Read the model definition and answer for the solid it produces. Units are mm, in the model's axes. Face numbers are marked on the shaded views. A direction names the side the tool comes from. Coordinates: 2 decimals unless noted, no trailing zeros. Loops run counter-clockwise (first coordinate to the right, second up) from the corner with the lowest first, then second, coordinate; pieces in that order, holes last.
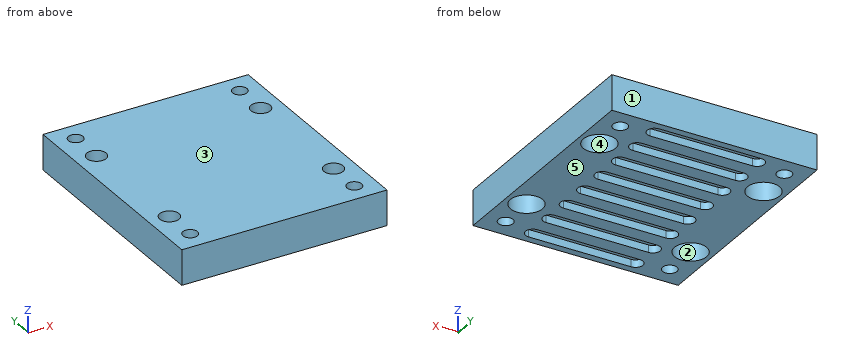
from build123d import *

# Parameters (mm, degrees)
SKETCH_1_W                     = 70
SKETCH_1_H                     = 80
EXTRUDE_1_DEPTH                = 12
HOLE_WIZARD_M6_1_D             = 5
HOLE_WIZARD_M6_1_2_D           = 6.6
HOLE_WIZARD_M6_1_2_CBORE_D     = 11
HOLE_WIZARD_M6_1_2_CBORE_DEPTH = 6.4
CUT_EXTRUDE_1_DEPTH            = 2.5
PATTERN_LINEAR_1_COUNT         = 8
PATTERN_LINEAR_1_PITCH         = 10


with BuildPart() as part:
    # 草图1 → 凸台-拉伸1 (new body)
    with BuildSketch(Plane.XY):
        Rectangle(SKETCH_1_W, SKETCH_1_H)
    extrude(amount=EXTRUDE_1_DEPTH)

    # Hole Wizard M6 _1 (through all)
    with Locations(Plane(origin=(0, 0, 0), x_dir=(-1, 0, 0), z_dir=(0, 0, -1))):
        with Locations((-28, -33), (-28, 33), (28, 33), (28, -33)):
            Hole(HOLE_WIZARD_M6_1_D / 2)

    # Hole Wizard M6 _1 2 (through all)
    with Locations(Plane(origin=(0, 0, 0), x_dir=(-1, 0, 0), z_dir=(0, 0, -1))):
        with Locations((-28, -21), (-28, 21), (28, -21), (28, 21)):
            CounterBoreHole(HOLE_WIZARD_M6_1_2_D / 2, HOLE_WIZARD_M6_1_2_CBORE_D / 2, HOLE_WIZARD_M6_1_2_CBORE_DEPTH)

    # 草图6 → 切除-拉伸1 (cut)
    with BuildSketch(Plane(origin=(0, 0, 0), x_dir=(-1, 0, 0), z_dir=(0, 0, -1))):
        with BuildLine():
            Line((17.5, 32.5), (-17.5, 32.5))
            ThreePointArc((-17.5, 32.5), (-20, 35), (-17.5, 37.5))
            Line((-17.5, 37.5), (17.5, 37.5))
            ThreePointArc((17.5, 37.5), (20, 35), (17.5, 32.5))
        make_face()
    cut_extrude_1 = extrude(amount=-CUT_EXTRUDE_1_DEPTH, mode=Mode.SUBTRACT)

    # 阵列(线性)1: 切除-拉伸1 ×8
    with Locations(*[(0, -i * PATTERN_LINEAR_1_PITCH, 0) for i in range(1, PATTERN_LINEAR_1_COUNT)]):
        add(cut_extrude_1, mode=Mode.SUBTRACT)


solid = part.part
Q1. Flat-ended cylindrical pins translate along their axes: pin 1 Ø2.5 at (x, y) = (7, 24) entering from -Z; pin 2 Ø3 at (x, y) = (28, 33) entering from -Z. Find the tip coordinate at first contact, or state that the pin passes through.
Findings below:
pin 1: stops at z = 2.5
pin 2: passes through
Q2. Which of the six approach directions +Z, -Z, +X, -X, +Y, -Y give full straight-line access (tool end or side, diameter ignored) to the marked faces 4 and 5?
Findings below:
face 4: -Z
face 5: -Z, +X, -X, +Y, -Y
Q3. A cutting plane is placed at B-B (x = 28). Give the vertices of the cut face in (y, z).
Findings below:
outline: (-40, 0) - (-35.5, 0) - (-35.5, 12) - (-40, 12) - close; (-30.5, 0) - (-26.5, 0) - (-26.5, 6.4) - (-24.3, 6.4) - (-24.3, 12) - (-30.5, 12) - close; (-17.7, 6.4) - (-15.5, 6.4) - (-15.5, 0) - (15.5, 0) - (15.5, 6.4) - (17.7, 6.4) - (17.7, 12) - (-17.7, 12) - close; (24.3, 6.4) - (26.5, 6.4) - (26.5, 0) - (30.5, 0) - (30.5, 12) - (24.3, 12) - close; (35.5, 0) - (40, 0) - (40, 12) - (35.5, 12) - close
Q4. Straight lines are drawn through the part: probe 1 along Y at (x, z) = (28, 10.45); probe 2 along Y at (x, z) = (-28, 2); probe 3 along X at (y, z) = (16.5, 6). For each, find the intervals that lie inside material, in ascending order.
Findings below:
probe 1: y = -40 to -35.5, -30.5 to -24.3, -17.7 to 17.7, 24.3 to 30.5, 35.5 to 40
probe 2: y = -40 to -35.5, -30.5 to -26.5, -15.5 to 15.5, 26.5 to 30.5, 35.5 to 40
probe 3: x = -35 to -31.16, -24.84 to 24.84, 31.16 to 35
Q5. Determine the mould class of the marked faces 1, 2 and 3 for opening direction Y: +Y half, -Y half, draft (parallel to the pull), parting line (faces both ways), or undercut.
Findings below:
face 1: +Y half
face 2: undercut
face 3: draft
Q6. A cutting plane is placed at A-A (z = 7.5). Count the separate pieces of the cut face and the enclosed holes in it, then the cut area to 3 significant figures.
Findings below:
separate pieces: 1
enclosed holes: 8
area: 5,380 mm2
Q7. A cutting plane is placed at C-C (y = -21). Give the vertices of the cut face in (x, z).
Findings below:
outline: (-35, 0) - (-33.5, 0) - (-33.5, 6.4) - (-31.3, 6.4) - (-31.3, 12) - (-35, 12) - close; (-24.7, 6.4) - (-22.5, 6.4) - (-22.5, 0) - (22.5, 0) - (22.5, 6.4) - (24.7, 6.4) - (24.7, 12) - (-24.7, 12) - close; (31.3, 6.4) - (33.5, 6.4) - (33.5, 0) - (35, 0) - (35, 12) - (31.3, 12) - close
